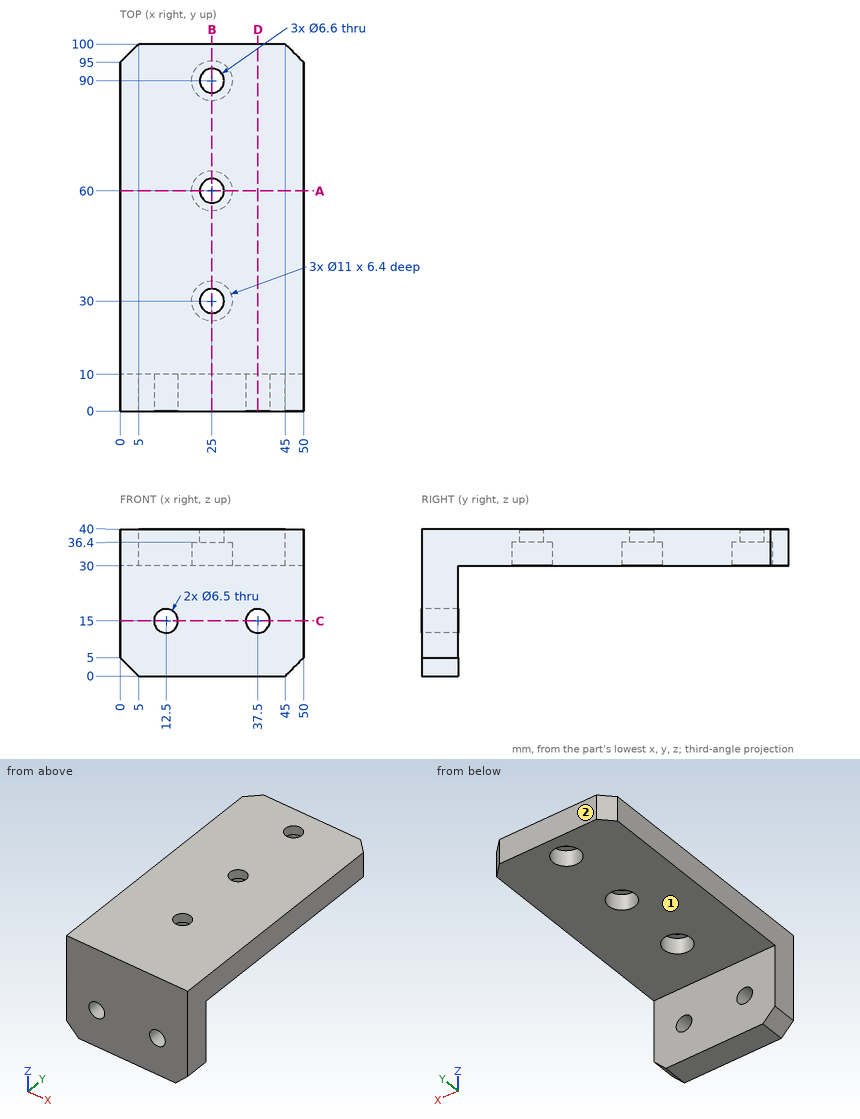
Geometry check sheet. Reference: drawing and pictorial views, mm from the part's lowest x, y, z. A direction names the side the tool comes from. Round coordinates to 2 decimals unless told otherwise and drop trailing zeros. Loops run counter-clockwise (first coordinate to the right, second up) from the corner with the lowest first, then second, coordinate; pieces in that order, holes last. Notation, with made-up numbers: (33.5, 84.25) -> (87.5, 84.25) arc R16 cw to (87.5, 97.25) -> close; hole circle Ø9 at (7, 60). An arc over 180 degrees is marked (long way). Use a Markdown table: item, result.
(1) Sectioned sample at C-C (z = 15). Enter the section's corners in (x, y), then the cut area to 3 significant figures.
Calculated:
| item | result |
|---|---|
| outline | (0, 0) -> (9.25, 0) -> (9.25, 10) -> (0, 10) -> close; (15.75, 0) -> (34.25, 0) -> (34.25, 10) -> (15.75, 10) -> close; (40.75, 0) -> (50, 0) -> (50, 10) -> (40.75, 10) -> close |
| area | 370 mm² |
(2) Sectioned sample at A-A (y = 60). Enter the section's corners in (x, z).
Calculated:
| item | result |
|---|---|
| outline | (0, 30) -> (19.5, 30) -> (19.5, 36.4) -> (21.7, 36.4) -> (21.7, 40) -> (0, 40) -> close; (28.3, 36.4) -> (30.5, 36.4) -> (30.5, 30) -> (50, 30) -> (50, 40) -> (28.3, 40) -> close |
(3) Set-up check for the marked faces 1 and 2: record each of +Z, -Z, +X, -X, +Y, -Y from which the full face is reachable in a straight line by a thin tool's end or side.
Calculated:
| item | result |
|---|---|
| face 1 | -Z, +X, -X, +Y |
| face 2 | +Z, -Z, +X, -X, +Y |
(4) Sectioned sample at D-D (x = 37.5). Enter the section's corners in (y, z), then the cut area to 4 significant figures.
Calculated:
| item | result |
|---|---|
| outline | (0, 0) -> (10, 0) -> (10, 11.75) -> (0, 11.75) -> close; (0, 18.25) -> (10, 18.25) -> (10, 30) -> (100, 30) -> (100, 40) -> (0, 40) -> close |
| area | 1,235 mm² |
(5) Scan lines: probe 1 along X at (y, z) = (5, 15); probe 2 along Y at (x, z) = (25, 35.25); probe 3 along Y at (x, z) = (22.5, 32). Record each from-to range of solid material in increasing order.
Calculated:
| item | result |
|---|---|
| probe 1 | 0 to 9.25, 15.75 to 34.25, 40.75 to 50 |
| probe 2 | 0 to 24.5, 35.5 to 54.5, 65.5 to 84.5, 95.5 to 100 |
| probe 3 | 0 to 25.1, 34.9 to 55.1, 64.9 to 85.1, 94.9 to 100 |
(6) Go/stop test with flat-tipped pins: P1, Ø12.5, axis at x = 25, y = 30, coming from the -Z side; P2, Ø10.5, axis at x = 25, y = 30, coming from the -Z side; P3, Ø17.5, axis at x = 25, y = 90, coming from the +Z side; P4, Ø10, axis at x = 37, z = 5.5, coming from the +Y side. Record where each tip stops, or that it passes through.
Calculated:
| item | result |
|---|---|
| P1 | z = 30 |
| P2 | z = 36.4 |
| P3 | z = 40 |
| P4 | y = 10 |
(7) Sectioned sample at B-B (x = 25). Give the number of separate pieces and of enclosed holes in the cut face, then the cut area to 3 significant figures.
Calculated:
| item | result |
|---|---|
| separate pieces | 4 |
| enclosed holes | 0 |
| area | 1,020 mm² |
